For this review, take the finished solid that the model builds, in its own axes (mm). A direction names the side the tool comes from. Coordinates: 2 decimals unless noted, no trailing zeros. Write each loop counter-clockwise with the first axis right and the second up, starting at its lowest first coordinate (ties: lowest second). Pieces come first, ordered by that corner, then holes. Notation, with made-up numbers: M -3.75,49.5 L 51.25,49.5 A27 cw 51.25,69.5 Z; hole C 84,60.5 d4. An arc over 180 degrees is marked long. Return JSON: item names as keys, results as strings.
```python
from build123d import *

# Parameters (mm, degrees)
EXTRUDE_358_DEPTH = 2.8
SKETCH_4_W        = 0.4
SKETCH_4_H        = 10.541451884
CHAMFER_1889_SIZE = 0.56
FILLET_1942_R     = 0.2


with BuildPart() as part:
    # 草图1 → Extrude 358 (new body)
    with BuildSketch(Plane(origin=(0, 0, 0), x_dir=(0, 0, -1), z_dir=(1, 0, 0))):
        Polygon((3.5, 2.020725942), (3.5, -2.020725942), (0, -4.041451884), (-3.5, -2.020725942), (-3.5, 2.020725942), (0, 4.041451884), align=None)
    extrude(amount=EXTRUDE_358_DEPTH)

    # 草图2 → 凸台-旋转1 (revolve)
    with BuildSketch(Plane.XY, mode=Mode.PRIVATE) as revolve_1_sk:
        Polygon((0, 0), (17.8, 0), (17.8, 1.3938), (17.8, 2), (0, 2), align=None)
    revolve(revolve_1_sk.sketch.rotate(Axis((0, 0, 0), (1, 0, 0)), 90), axis=Axis((0, 0, 0), (1, 0, 0)))

    # 草图3 → 切除-旋转1 (revolve, cut)
    with BuildSketch(Plane.XY):
        Polygon((0, 3.5), (3.199358737, 9.041451884), (3.199358737, 14.041451884), (-10, 14.041451884), (-10, 3.5), align=None)
    revolve(axis=Axis((0, 0, 0), (1, 0, 0)), mode=Mode.SUBTRACT)

    # 草图5 → 切除-旋转2 (revolve, cut)
    with BuildSketch(Plane.XY):
        Polygon((2.8, 3.5), (-0.399358737, 9.041451884), (-0.399358737, 14.041451884), (9.600641263, 14.041451884), (9.600641263, 3.5), align=None)
    revolve(axis=Axis((0, 0, 0), (1, 0, 0)), mode=Mode.SUBTRACT)

    # 草图4 → 切除-旋转3 (revolve, cut)
    with BuildSketch(Plane.XY, mode=Mode.PRIVATE) as cut_revolve_3_sk:
        with Locations((2.6, 8.770725942)):
            Rectangle(SKETCH_4_W, SKETCH_4_H)
    revolve(cut_revolve_3_sk.sketch.rotate(Axis((0, 0, 0), (1, 0, 0)), 270), axis=Axis((0, 0, 0), (1, 0, 0)), mode=Mode.SUBTRACT)

    # Chamfer 1889
    chamfer_1889_edges = [part.edges().sort_by_distance(p)[0] for p in [
        (17.8, 0, -2),
    ]]
    chamfer(chamfer_1889_edges, length=CHAMFER_1889_SIZE)

    # Fillet 1942
    fillet_1942_edges = [part.edges().sort_by_distance(p)[0] for p in [
        (2.8, 0, -2),
    ]]
    fillet(fillet_1942_edges, radius=FILLET_1942_R)


solid = part.part
```
1. For faces 1 (the face through (2.4, -1.8, 3.2)), 2 (the face through (2.4, -1.85, -3.15)), 3 (the face through (10, 2, 0)), list the 3-axis set-ups (+Z, -Z, +X, -X, +Y, -Y) from which the entire face can be reached by the end or side of a thin tool; tool diameter is ignored.
Checks:
{"face 1": "+Z, +X, -Y", "face 2": "-Z, +X, -Y", "face 3": "+X"}
2. We need section A-A (x = 14). State the section outline as (y, z) points.
Checks:
{"outline": "C 0,0 d4"}
3. Clearance check with flat-ended pins moving along their axes: pin 1 Ø1.4 at (y, z) = (1, 3) entering from +X; pin 2 Ø0.8 at (y, z) = (4, 1) entering from +X; pin 3 Ø1 at (x, y) = (11, -2) entering from +Z; pin 4 Ø2 at (x, y) = (4.5, 2.5) entering from -Z. State where each tip first meets the part, or that it passes through.
Checks:
{"pin 1": "x = 2.8", "pin 2": "through", "pin 3": "z = 1.32", "pin 4": "z = -1.32"}
4. Wall thickness on L1, parallel to X at y = -2.25, z = -0.5; L2, parallel to Y at x = 2, z = -0.5; L3, parallel to X at y = 3.5, z = -0.5: over which ranges is each line inside the solid? List them lowest first. Write a range as from..to.
Checks:
{"L1": "0..2.8", "L2": "-3.75..3.75", "L3": "0.02..2.4"}
